Part print with two shaded views. Sizes in mm from the minimum x, y, z corner. A direction names the side the tool comes from. Give positions to 0.01 mm unless a question says otherwise; leave off trailing zeros. Write each loop counter-clockwise with the first axis right and the second up, starting at its lowest first coordinate (ties: lowest second). Pieces come first, ordered by that corner, then holes.
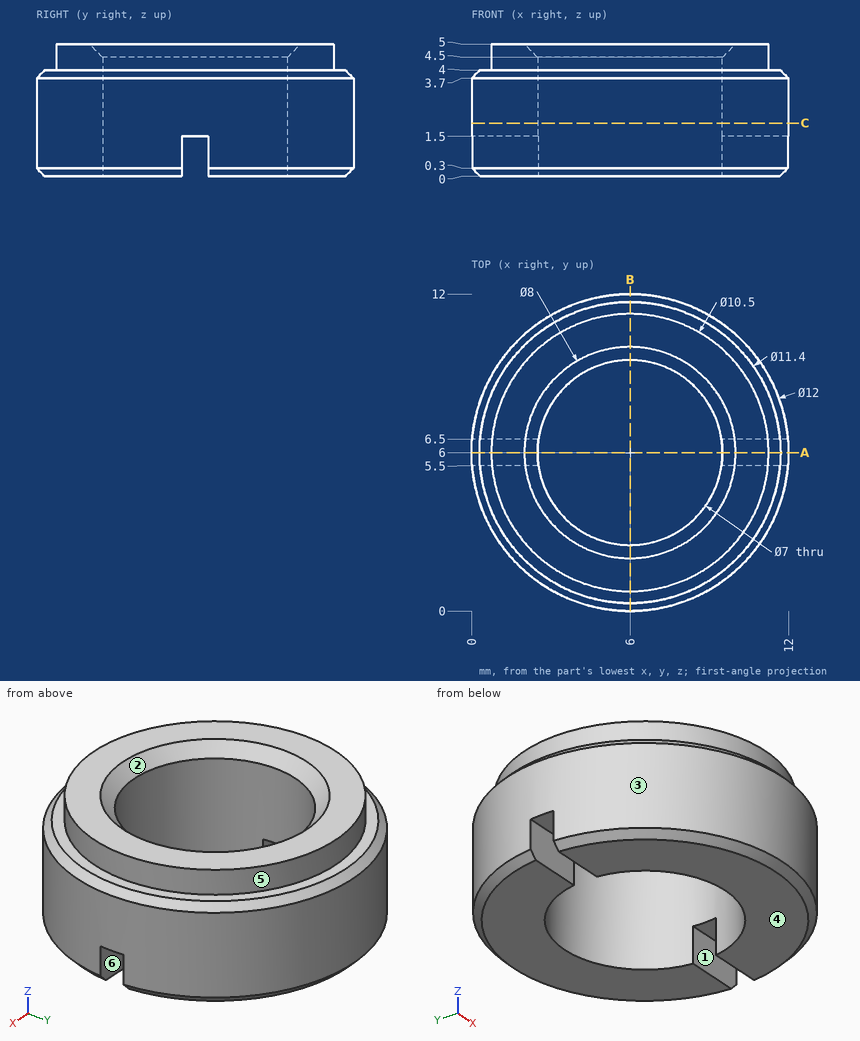
1) Saw through at C-C (z = 2). Write the cut outline in (x, y).
Check result:
outline: circle Ø12 at (6, 6); hole circle Ø7 at (6, 6)
2) Flat gauge pins, fed straight in: P1, Ø4, axis at x = 6, y = 6, coming from the +Z side; P2, Ø0.8, axis at x = 1, z = 0.5, coming from the -Y side; P3, Ø2, axis at y = 3.5, z = 4, coming from the +X side; P4, Ø1.7, axis at x = 11, z = 1, coming from the +Y side. Where does each tip first touch, or does it go through?
Check result:
P1: passes through
P2: stops at y = 2.15
P3: stops at x = 11.8
P4: stops at y = 10.33
3) Saw through at A-A (y = 6). Write the cut outline in (x, z).
Check result:
outline: (0, 1.5) - (2.5, 1.5) - (2.5, 4.5) - (2, 5) - (0.75, 5) - (0.75, 4) - (0.3, 4) - (0, 3.7) - close; (9.5, 1.5) - (12, 1.5) - (12, 3.7) - (11.7, 4) - (11.25, 4) - (11.25, 5) - (10, 5) - (9.5, 4.5) - close
4) Saw through at B-B (x = 6). Write the cut outline in (y, z), and give its area (3 significant figures).
Check result:
outline: (0, 0.3) - (0.3, 0) - (2.5, 0) - (2.5, 4.5) - (2, 5) - (0.75, 5) - (0.75, 4) - (0.3, 4) - (0, 3.7) - close; (9.5, 0) - (11.7, 0) - (12, 0.3) - (12, 3.7) - (11.7, 4) - (11.25, 4) - (11.25, 5) - (10, 5) - (9.5, 4.5) - close
area: 23.1 mm2
5) 3-axis set-ups, long thin cutter, end or side, ignore diameter. For the marked faces 4, 5 and 6: which of +Z, -Z, +X, -X, +Y, -Y reach the whole face in a straight line?
Check result:
face 4: -Z, +X, -X, +Y, -Y
face 5: +Z
face 6: -Z, +X, -X
6) Drill centre lines: L1, parallel to X at y = 6, z = 2.85; L2, parallel to Z at x = 1.5, y = 3. Where is each one in solid material? Low to high.
Check result:
L1: x = 0 to 2.5, 9.5 to 12
L2: z = 0 to 4
7) Mould opens along X. For the marked faces 1, 2 and 3 say: +X half, -X half, draft (parallel to the pull), parting line (faces both ways), or undercut.
Check result:
face 1: draft
face 2: undercut
face 3: parting line
